Geometry: see drawing. Coordinates: mm, zero at the bounding-box minimum. A direction names the side the tool comes from. Round coordinates to 2 decimals unless told otherwise and drop trailing zeros. Loops run counter-clockwise (first coordinate to the right, second up) from the corner with the lowest first, then second, coordinate; pieces in that order, holes last.
(1) Access query for the marked faces 1 and 2. Directions: +Z, -Z, +X, -X, +Y, -Y. A direction counts if a zero-diameter tool reaches every point of the face in a straight line with its end or side. Return the directions, or none.
(2) Line query: line 1 (X direction, y = 4, z = 3.5); line 2 (Y direction, x = 14, z = 2.5); line 3 (Z direction, x = 9, y = 3.5). Output: solid intervals per line, ascending.
(3) Cut plane B-B, the plane x = 9. Output: boundary loops of the cut face in (y, z), and give its area (3 significant figures).
(4) First-contact query: pin 1 Ø2 at (x, y) = (4, 4) entering from +Z; pin 2 Ø5.5 at (x, z) = (13.5, 16) entering from -Y. Flat tips, straight axial feed; report the tip coordinate or a pass-through.
(5) Cut plane C-C, the plane z = 20.5. Output: boundary loops of the cut face in (x, y), and give its area (3 significant figures).
(6) Cut plane A-A, the plane z = 5.5. Output: boundary loops of the cut face in (x, y), and give its area (3 significant figures).
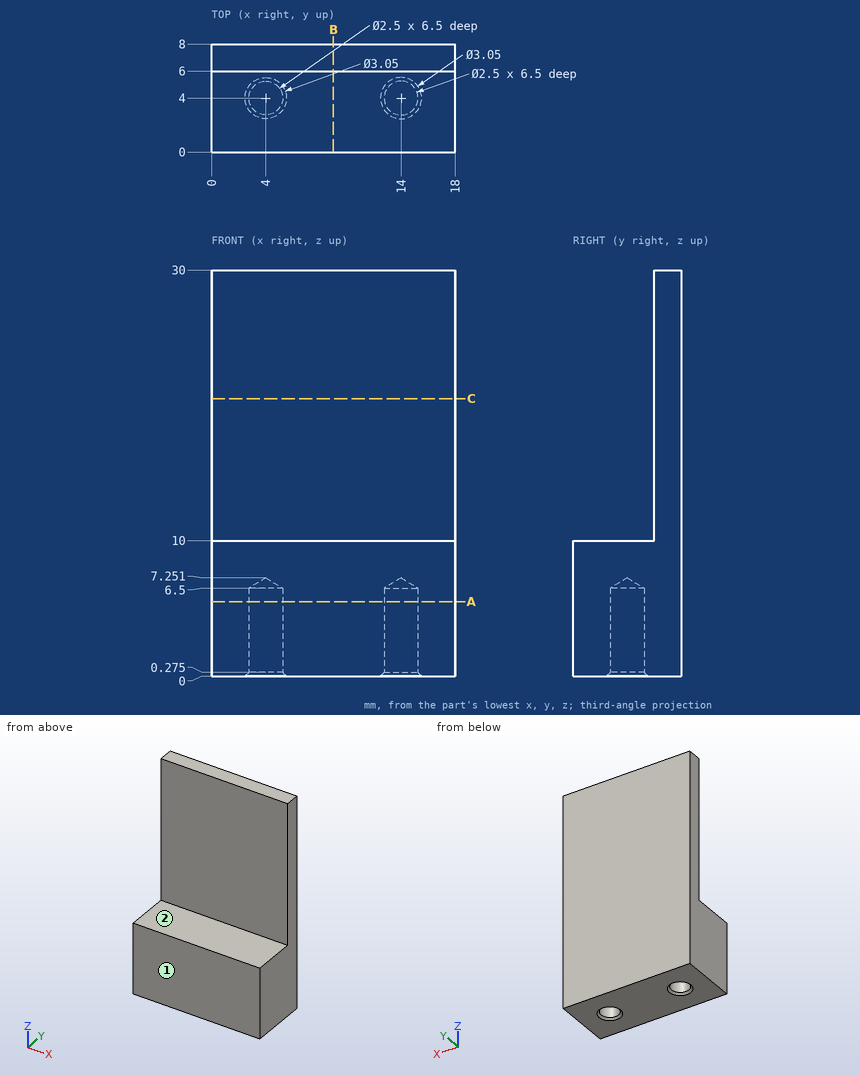
Reported:
1. face 1: +Z, -Z, +X, -X, -Y
1. face 2: +Z, +X, -X, -Y
2. line 1: x = 0 to 2.75, 5.25 to 12.75, 15.25 to 18
2. line 2: y = 0 to 2.75, 5.25 to 8
2. line 3: z = 0 to 10
3. outline: (0, 0) - (8, 0) - (8, 30) - (6, 30) - (6, 10) - (0, 10) - close
3. area: 120 mm2
4. pin 1: stops at z = 10
4. pin 2: stops at y = 6
5. outline: (0, 6) - (18, 6) - (18, 8) - (0, 8) - close
5. area: 36.0 mm2
6. outline: (0, 0) - (18, 0) - (18, 8) - (0, 8) - close; hole circle Ø2.5 at (4, 4); hole circle Ø2.5 at (14, 4)
6. area: 134 mm2
